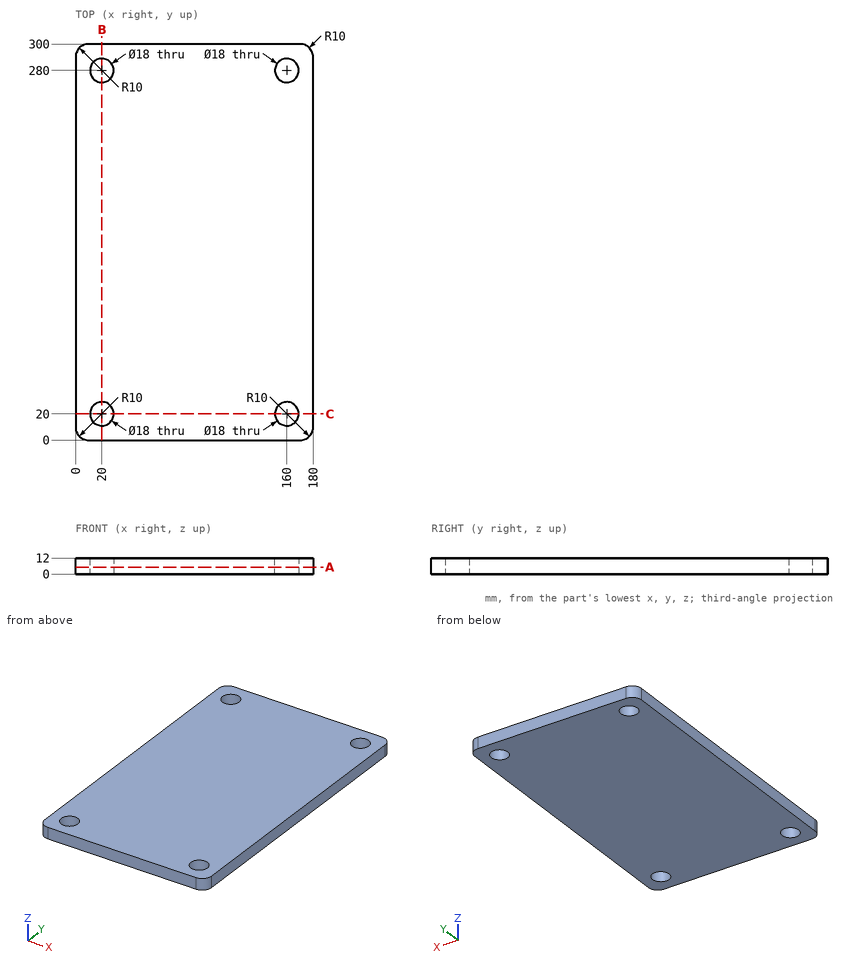
Print and shaded views of the part. All mm, measured from the part's lowest x, y and z. Round coordinates to 2 decimals unless told otherwise and drop trailing zeros. Write each loop counter-clockwise with the first axis right and the second up, starting at its lowest first coordinate (ties: lowest second). Pieces come first, ordered by that corner, then holes. Notation, with made-up numbers: (65, 18.5) - (69, 18.5) arc R15 ccw to (69, 30.5) - close; hole circle Ø1 at (14.5, 62.5). An arc over 180 degrees is marked (long way). Write each question's results on one line, items separated by ' | '. Start each with the question number.
Item 1: Saw through at A-A (z = 5.25). Write the cut outline in (x, y), and give its area (3 significant figures).
Item 2: Saw through at C-C (y = 20). Write the cut outline in (x, z).
Item 3: Saw through at B-B (x = 20). Write the cut outline in (y, z), and give its area (3 significant figures).
Item 4: Wall check: L1, parallel to Y at x = 20, z = 9.25; L2, parallel to X at y = 280, z = 5.5; L3, parallel to Y at x = 156.5, z = 5. Give the ranges that are in metal, low to high. Write a range as [from, to].
Results are:
1) outline: (0, 10) arc R10 ccw to (10, 0) - (170, 0) arc R10 ccw to (180, 10) - (180, 290) arc R10 ccw to (170, 300) - (10, 300) arc R10 ccw to (0, 290) - close; hole circle Ø18 at (20, 20); hole circle Ø18 at (20, 280); hole circle Ø18 at (160, 20); hole circle Ø18 at (160, 280) | area: 52,900 mm²
2) outline: (0, 0) - (11, 0) - (11, 12) - (0, 12) - close; (29, 0) - (151, 0) - (151, 12) - (29, 12) - close; (169, 0) - (180, 0) - (180, 12) - (169, 12) - close
3) outline: (0, 0) - (11, 0) - (11, 12) - (0, 12) - close; (29, 0) - (271, 0) - (271, 12) - (29, 12) - close; (289, 0) - (300, 0) - (300, 12) - (289, 12) - close | area: 3,170 mm²
4) L1: y = [0, 11], [29, 271], [289, 300] | L2: x = [0, 11], [29, 151], [169, 180] | L3: y = [0, 11.71], [28.29, 271.71], [288.29, 300]
